Read the model definition and answer for the solid it produces. Units are mm, in the model's axes. Face numbers are marked on the shaded views. Coordinates: 2 decimals unless noted, no trailing zeros. Order: outer loops, then holes, each group sorted by start corner. A loop starts at its lowest first (then second) coordinate and runs counter-clockwise, first axis right, second up. Notation, with made-up numbers: (58.25, -32) -> (93.25, -32) arc R22 cw to (93.25, -15) -> close; hole circle Ø7 at (-4.75, -38). An arc over 180 degrees is marked (long way). Use CSV: the item, a comma, the result in double quotes.
```python
from build123d import *

# Parameters (mm, degrees)
SKETCH1_R           = 3.175
SKETCH1_R_2         = 25
BOSS_EXTRUDE1_DEPTH = 10
SKETCH2_R           = 3.175
CUT_EXTRUDE1_DEPTH  = 3
SCALE_RATIO_1_SCALE = 1.3


with BuildPart() as part:
    # Sketch1 → Boss-Extrude1 (new body)
    with BuildSketch(Plane.XY):
        with BuildLine():
            Line((-52.990381057, -15.594010768), (-12.990381057, 53.688021535))
            ThreePointArc((-12.990381057, 53.688021535), (0, 61.188021535), (12.990381057, 53.688021535))
            Line((12.990381057, 53.688021535), (52.990381057, -15.594010768))
            ThreePointArc((52.990381057, -15.594010768), (52.990381057, -30.594010768), (40, -38.094010768))
            Line((40, -38.094010768), (-40, -38.094010768))
            ThreePointArc((-40, -38.094010768), (-52.990381057, -30.594010768), (-52.990381057, -15.594010768))
        make_face()
        with Locations((-40, -23.094010768)):
            Circle(SKETCH1_R, mode=Mode.SUBTRACT)
        with Locations((40, -23.094010768)):
            Circle(SKETCH1_R, mode=Mode.SUBTRACT)
        with Locations((0, 46.188021535)):
            Circle(SKETCH1_R, mode=Mode.SUBTRACT)
        Circle(SKETCH1_R_2, mode=Mode.SUBTRACT)
    extrude(amount=BOSS_EXTRUDE1_DEPTH)

    # Sketch2 → Cut-Extrude1 (cut)
    # profile 1 of 3: a face of its own
    with BuildSketch(Plane.XY):
        with BuildLine():
            Line((-39.68174609, -27.58274271), (-46.857480139, -28.091506755))
            ThreePointArc((-46.857480139, -28.091506755), (-47.794228634, -27.594010768), (-47.75669855, -26.53401478))
            Line((-47.75669855, -26.53401478), (-43.728228938, -20.574028825))
            ThreePointArc((-43.728228938, -20.574028825), (-36.102885683, -20.844010768), (-39.68174609, -27.58274271))
        make_face()
        with Locations((-40, -23.094010768)):
            Circle(SKETCH2_R, mode=Mode.SUBTRACT)
    # profile 2 of 3: a face of its own
    with BuildSketch(Plane.XY):
        with BuildLine():
            Line((-4.046482848, 48.156771535), (-0.899218411, 54.625521535))
            ThreePointArc((-0.899218411, 54.625521535), (0, 55.188021535), (0.899218411, 54.625521535))
            Line((0.899218411, 54.625521535), (4.046482848, 48.156771535))
            ThreePointArc((4.046482848, 48.156771535), (0, 41.688021535), (-4.046482848, 48.156771535))
        make_face()
        with Locations((0, 46.188021535)):
            Circle(SKETCH2_R, mode=Mode.SUBTRACT)
    # profile 3 of 3: a face of its own
    with BuildSketch(Plane.XY):
        with BuildLine():
            Line((43.728228938, -20.574028825), (47.75669855, -26.53401478))
            ThreePointArc((47.75669855, -26.53401478), (47.794228634, -27.594010768), (46.857480139, -28.091506755))
            Line((46.857480139, -28.091506755), (39.68174609, -27.58274271))
            ThreePointArc((39.68174609, -27.58274271), (36.102885683, -20.844010768), (43.728228938, -20.574028825))
        make_face()
        with Locations((40, -23.094010768)):
            Circle(SKETCH2_R, mode=Mode.SUBTRACT)
    extrude(amount=CUT_EXTRUDE1_DEPTH, mode=Mode.SUBTRACT)


with BuildPart() as part_1:
    # Scale ratio 1: scaled about (0, 0, 0)
    add(part.part.scale(SCALE_RATIO_1_SCALE))


solid = part_1.part
```
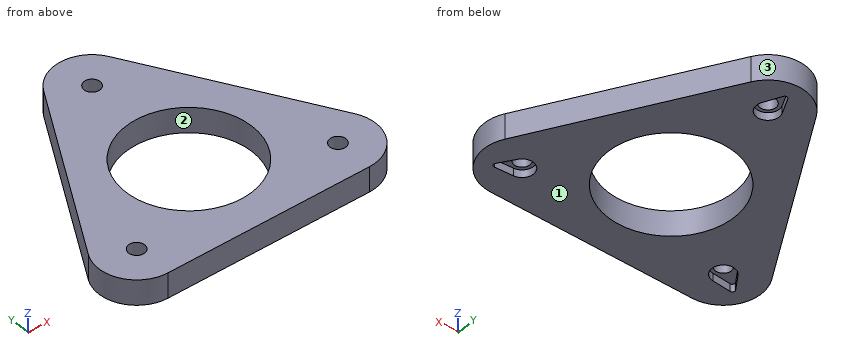
Item 1: Straight lines are drawn through the part: line 1 along Y through (x, z) = (17, 6); line 2 along X through (y, z) = (-33, 7.5); line 3 along Y through (x, z) = (-61.5, 1). For each, find the intervals that lie inside material, in ascending order.
Return value:
line 1,"y = -49.52 to -27.7, 27.7 to 69.6"
line 2,"x = -71.27 to -54.86, -49.14 to 49.14, 54.86 to 71.27"
line 3,"y = -47.05 to -36.42, -33.63 to -7.48"
Item 2: Find section A-A, the plane x = -8. Give the vertices of the cut face in (y, z), then the cut area to 3 significant figures.
Return value:
outline,"(-49.52, 0) -> (-31.5, 0) -> (-31.5, 13) -> (-49.52, 13) -> close; (31.5, 0) -> (77.83, 0) -> (77.83, 13) -> (31.5, 13) -> close"
area,"837 mm^2"
Item 3: Find section B-B, the plane y = 27.5. Give the vertices of the cut face in (x, z), then the cut area to 3 significant figures.
Return value:
outline,"(-41.31, 0) -> (-17.32, 0) -> (-17.32, 13) -> (-41.31, 13) -> close; (17.32, 0) -> (41.31, 0) -> (41.31, 13) -> (17.32, 13) -> close"
area,"624 mm^2"
Item 4: The mould has two halves that part along X. Classify the marked faces 1, 2 and 3: +X half, -X half, draft (parallel to the pull), parting line (faces both ways), or undercut.
Return value:
face 1,"draft"
face 2,"undercut"
face 3,"parting line"
Item 5: Find section C-C, the plane z = 5.75. Give the vertices of the cut face in (x, y) (1 decimal).
Return value:
outline,"(-68.9, -20.3) arc R19.5 ccw to (-52, -49.5) -> (52, -49.5) arc R19.5 ccw to (68.9, -20.3) -> (16.9, 69.8) arc R19.5 ccw to (-16.9, 69.8) -> close; hole circle Ø8.3 at (-52, -30); hole circle Ø65 at (0, 0); hole circle Ø8.3 at (0, 60); hole circle Ø8.3 at (52, -30)"
Item 6: Each of these flat-tipped pins is pushed along its axis until it touches: P1, Ø5, axis at y = 4, z = 7, coming from the +X side; P2, Ø2, axis at y = 9.5, z = 4, coming from the -X side; P3, Ø5, axis at y = -21, z = 5.5, coming from the +X side. Where does it stop, or does it pass through?
Return value:
P1,"stops at x = 56.32"
P2,"stops at x = -52.28"
P3,"stops at x = 70.38"
